Geometry: final body of the model. Coordinates: model frame, mm. A direction names the side the tool comes from. Give positions to 0.01 mm unless a question says otherwise; leave off trailing zeros. Write each loop counter-clockwise with the first axis right and the second up, starting at its lowest first coordinate (ties: lowest second). Pieces come first, ordered by that corner, then holes.
from build123d import *

# Parameters (mm, degrees)
SKETCH1_R           = 180
BOSS_EXTRUDE1_DEPTH = 100
SKETCH2_R           = 25
CUT_EXTRUDE1_DEPTH  = 80
SKETCH3_W           = 150
SKETCH3_H           = 62.418974348
BOSS_EXTRUDE3_DEPTH = 50
BOSS_EXTRUDE4_START = -15
SKETCH4_R           = 215
SKETCH4_R_2         = 180
SKETCH4_R_3         = 5.5
BOSS_EXTRUDE4_DEPTH = 15
CHAMFER1_SIZE       = 5
BOSS_EXTRUDE5_START = 150
SKETCH5_W           = 170
SKETCH5_H           = 200
BOSS_EXTRUDE5_DEPTH = 50


with BuildPart() as part:
    # Sketch1 → Boss-Extrude1 (new, symmetric)
    with BuildSketch(Plane.XY):
        Circle(SKETCH1_R)
    extrude(amount=BOSS_EXTRUDE1_DEPTH, both=True)

    # Sketch2 → Cut-Extrude1 (cut)
    with BuildSketch(Plane(origin=(0, 0, -100), x_dir=(-1, 0, 0), z_dir=(0, 0, -1))):
        Circle(SKETCH2_R)
    extrude(amount=-CUT_EXTRUDE1_DEPTH, mode=Mode.SUBTRACT)

    # Sketch3 → Boss-Extrude3 (add)
    with BuildSketch(Plane.XY.offset(100)):
        with Locations((0, 168.790512826)):
            Rectangle(SKETCH3_W, SKETCH3_H)
    extrude(amount=-BOSS_EXTRUDE3_DEPTH)

    # Sketch4 → Boss-Extrude4 (add)
    with BuildSketch(Plane(origin=(0, 0, -100), x_dir=(-1, 0, 0), z_dir=(0, 0, -1)).offset(BOSS_EXTRUDE4_START)):
        Circle(SKETCH4_R)
        Circle(SKETCH4_R_2, mode=Mode.SUBTRACT)
        with Locations((-102.5, 177.535207776)):
            Circle(SKETCH4_R_3, mode=Mode.SUBTRACT)
        with Locations((102.5, 177.535207776)):
            Circle(SKETCH4_R_3, mode=Mode.SUBTRACT)
        with Locations((205, 0)):
            Circle(SKETCH4_R_3, mode=Mode.SUBTRACT)
        with Locations((102.5, -177.535207776)):
            Circle(SKETCH4_R_3, mode=Mode.SUBTRACT)
        with Locations((-102.5, -177.535207776)):
            Circle(SKETCH4_R_3, mode=Mode.SUBTRACT)
        with Locations((-205, 0)):
            Circle(SKETCH4_R_3, mode=Mode.SUBTRACT)
    extrude(amount=BOSS_EXTRUDE4_DEPTH)

    # Chamfer1
    chamfer1_edges = [part.edges().sort_by_distance(p)[0] for p in [
        (-97.211110476, -151.492574075, 100),
    ]]
    chamfer(chamfer1_edges, length=CHAMFER1_SIZE)

    # Sketch5 → Boss-Extrude5 (add)
    with BuildSketch(Plane(origin=(0, 0, 0), x_dir=(0, 0, -1), z_dir=(1, 0, 0)).offset(BOSS_EXTRUDE5_START)):
        Rectangle(SKETCH5_W, SKETCH5_H)
    boss_extrude5 = extrude(amount=BOSS_EXTRUDE5_DEPTH)

    # Mirror1: Boss-Extrude5 across plane
    add(boss_extrude5.mirror(Plane(origin=(0, 0, 0), x_dir=(0, 0, 1), z_dir=(1, 0, 0))))


solid = part.part
Q1. Ray query, line 1 along Y through (x, z) = (-102.5, -94); line 2 along X through (y, z) = (-0.5, -25) (3 decimals); line 3 along Y through (x, z) = (1, -45). Return the intervals inside material, ascending.
Filled sheet:
line 1: y = -188.99 to -183.04, -172.04 to 172.04, 183.04 to 188.99
line 2: x = -200 to -24.995, 24.995 to 200
line 3: y = -180 to -24.98, 24.98 to 180
Q2. Section C-C on z = 24. Output: boundary loops of the cut face in (x, y).
Filled sheet:
outline: (-200, -100) - (-150, -100) - (-150, -99.5) arc R180 ccw to (150, -99.5) - (150, -100) - (200, -100) - (200, 100) - (150, 100) - (150, 99.5) arc R180 ccw to (-150, 99.5) - (-150, 100) - (-200, 100) - close
Q3. Pin query (flat end, axial travel): P1, Ø3, axis at x = -128, z = -32, coming from the -Y side; P2, Ø5, axis at x = -172, y = -70.5, coming from the +Z side; P3, Ø12.5, axis at y = 175, z = 83, coming from the +X side. Return the tip coordinate at first contact, or that it passes through.
Filled sheet:
P1: stops at y = -128.05
P2: stops at z = 85
P3: stops at x = 75
Q4. Section B-B on x = 0. Output: boundary loops of the cut face in (y, z).
Filled sheet:
outline: (-215, -100) - (-25, -100) - (-25, -20) - (25, -20) - (25, -100) - (215, -100) - (215, -85) - (180, -85) - (180, 50) - (200, 50) - (200, 100) - (-175, 100) - (-180, 95) - (-180, -85) - (-215, -85) - close
Q5. Section D-D on x = 102.5. Count the separate pieces of the cut face and the enclosed holes in it, plus the area to 3 significant figures.
Filled sheet:
separate pieces: 3
enclosed holes: 0
area: 60,100 mm2
Q6. Access query for faces 1 (the flat face through (197, -94, -85)), 2 (the flat face through (211, 1, -85)), 3 (the cylindrical face through (-142.84, -109.53, 6.26)), 4 (the cylindrical face through (-23.846, 7.509, -60.56)). Directions: +Z, -Z, +X, -X, +Y, -Y. A direction counts if a zero-diameter tool reaches every point of the face in a straight line with its end or side. Return the directions, or none.
Filled sheet:
face 1: -Z, +X, -Y
face 2: +Z, +X, +Y, -Y
face 3: none
face 4: -Z
Q7. Pull-direction query (Y, two-part tool) for faces 5 (the cylindrical face through (-101.308, -182.904, -92.395)), 6 (the flat face through (-2, 15, 100)), 7 (the flat face through (-1, 200, 75)); classes: released by +Y, released by -Y, zero draft, split by the parting line, or undercut.
Filled sheet:
face 5: undercut
face 6: zero draft
face 7: released by +Y
Q8. Section A-A on z = -29. Output: boundary loops of the cut face in (x, y), plus the area to 3 significant figures.
Filled sheet:
outline: (-200, -100) - (-150, -100) - (-150, -99.5) arc R180 ccw to (150, -99.5) - (150, -100) - (200, -100) - (200, 100) - (150, 100) - (150, 99.5) arc R180 ccw to (-150, 99.5) - (-150, 100) - (-200, 100) - close; hole circle Ø50 at (0, 0)
area: 112,000 mm2
